Answer from the drawing. Dimensions are ordinates in mm from the lowest x, y and z of the part. A direction names the side the tool comes from. Coordinates: 2 decimals unless noted, no trailing zeros. Write each loop counter-clockwise with the first axis right and the second up, starting at its lowest first coordinate (ties: lowest second). Pieces come first, ordered by that corner, then holes. Notation, with made-up numbers: (-17.75, 17) -> (17.25, 17) arc R10 cw to (17.25, 28) -> close; hole circle Ø1 at (67.5, 66). An arc over 180 degrees is marked (long way). Answer as a JSON object with one key per item and string values. Group by question number.
(1) Find section C-C (z = 54.5). Give the vertices of the cut face in (x, y), then the cut area to 3 significant figures.
(2) Find section A-A (x = 24). Give the vertices of the cut face in (y, z), then the cut area to 3 significant figures.
(3) Which of the six approach directions +Z, -Z, +X, -X, +Y, -Y give full straight-line access (tool end or side, diameter ignored) to the marked faces 1 and 2?
(4) Find section D-D (z = 4). Give the vertices of the cut face in (x, y), then the cut area to 3 significant figures.
(5) Find section B-B (y = 54). Give the vertices of the cut face in (x, z).
(6) Flat-ended cylindrical pins translate along their axes: P1, Ø5, axis at x = 33, z = 32.5, coming from the +Y side; P2, Ø14.5, axis at x = 17.5, y = 45, coming from the +Z side; P3, Ø2.5, axis at x = 6, z = 10, coming from the +Y side. Find the tip coordinate at first contact, or state that the pin passes through.
(7) Straight lines are drawn through the part: L1, parallel to X at y = 55, z = 10; L2, parallel to X at y = 10, z = 57; L3, parallel to Y at x = 5, z = 56. For each, find the intervals that lie inside material, in ascending order.
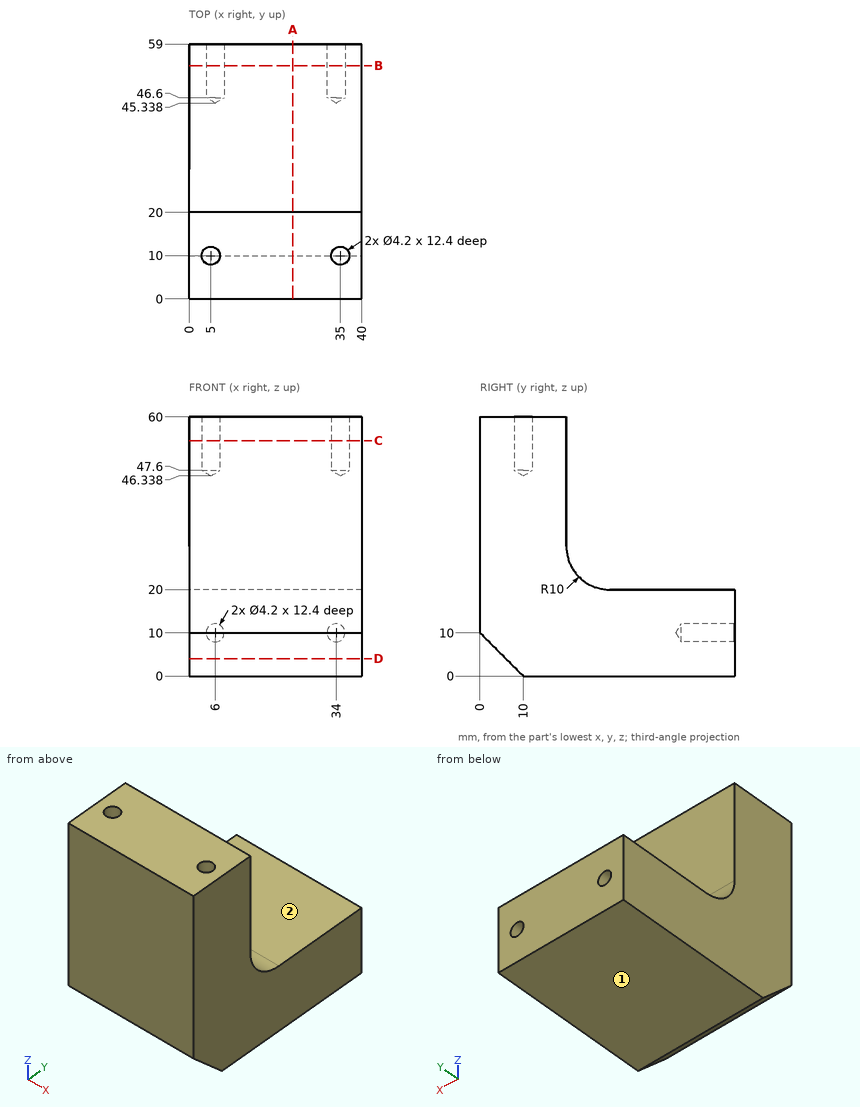
Results below:
{
 "1": {"outline": "(0, 0) -> (40, 0) -> (40, 20) -> (0, 20) -> close; hole circle Ø4.2 at (5, 10); hole circle Ø4.2 at (35, 10)", "area": "772 mm2"},
 "2": {"outline": "(0, 10) -> (10, 0) -> (59, 0) -> (59, 20) -> (30, 20) arc R10 cw to (20, 30) -> (20, 60) -> (0, 60) -> close", "area": "1,950 mm2"},
 "3": {"face 1": "-Z, +X, -X, +Y, -Y", "face 2": "+Z, +X, -X, +Y"},
 "4": {"outline": "(0, 6) -> (40, 6) -> (40, 59) -> (0, 59) -> close", "area": "2,120 mm2"},
 "5": {"outline": "(0, 0) -> (40, 0) -> (40, 20) -> (0, 20) -> close; hole circle Ø4.2 at (6, 10); hole circle Ø4.2 at (34, 10)"},
 "6": {"P1": "stops at y = 20", "P2": "stops at z = 20", "P3": "stops at y = 46.09"},
 "7": {"L1": "x = 0 to 3.9, 8.1 to 31.9, 36.1 to 40", "L2": "x = 0 to 2.9, 7.1 to 32.9, 37.1 to 40", "L3": "y = 0 to 7.9, 12.1 to 20"}
}
